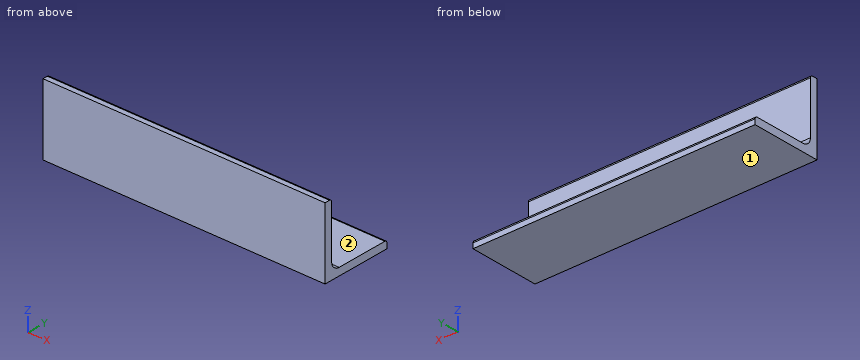
```python
from build123d import *

# Parameters (mm, degrees)
BASE_DEPTH = 300


with BuildPart() as part:
    # Sketch1 → Base (new body)
    with BuildSketch(Plane.YZ):
        with BuildLine():
            Line((0, 75), (0, 0))
            Line((0, 0), (75, 0))
            Line((75, 0), (75, 5.333333333))
            ThreePointArc((75, 5.333333333), (74.218951416, 7.218951416), (72.333333333, 8))
            Line((72.333333333, 8), (17, 8))
            ThreePointArc((17, 8), (10.636038969, 10.636038969), (8, 17))
            Line((8, 17), (8, 72.333333333))
            ThreePointArc((8, 72.333333333), (7.218951416, 74.218951416), (5.333333333, 75))
            Line((5.333333333, 75), (0, 75))
        make_face()
    extrude(amount=BASE_DEPTH)


solid = part.part
```
Geometry check sheet. Reference: the model listing, model coordinates, mm. Face numbers are marked on the shaded views. A direction names the side the tool comes from. Coordinates: 2 decimals unless noted, no trailing zeros. Loops run counter-clockwise (first coordinate to the right, second up) from the corner with the lowest first, then second, coordinate; pieces in that order, holes last. Notation, with made-up numbers: (61.25, 64.5) -> (87.25, 64.5) arc R16 cw to (87.25, 74.5) -> close; hole circle Ø9 at (48, -3). An arc over 180 degrees is marked (long way). Put each result on its own line as item: value.
1) Gauge pin test, flat ends, axial feed: pin 1 Ø5 at (x, z) = (50.5, 66.5) entering from +Y; pin 2 Ø12 at (y, z) = (14.5, 40) entering from +X. Record the tip position at first contact, or that the pin passes through.
Result set:
pin 1: stops at y = 8
pin 2: passes through
2) Cross-section at B-B on z = 63. Record the boundary of the cut face in (x, y), plus the area to 3 significant figures.
Result set:
outline: (0, 0) -> (300, 0) -> (300, 8) -> (0, 8) -> close
area: 2,400 mm^2
3) Tool access check on the marked faces 1 and 2. Record the directions out of +Z, -Z, +X, -X, +Y, -Y that give a thin tool (end or side, any length) a straight path to the whole face; none if there is none.
Result set:
face 1: -Z, +X, -X, +Y, -Y
face 2: +Z, +X, -X, +Y
4) Thickness scan on line 1 (Z direction, x = 95, y = 53.5); line 2 (Y direction, x = 210.5, z = 10.5). Record the ranges inside material, lowest first.
Result set:
line 1: z = 0 to 8
line 2: y = 0 to 10.78
5) Cross-section at A-A on x = 203.5. Record the boundary of the cut face in (y, z).
Result set:
outline: (0, 0) -> (75, 0) -> (75, 5.33) arc R2.67 ccw to (72.33, 8) -> (17, 8) arc R9 cw to (8, 17) -> (8, 72.33) arc R2.67 ccw to (5.33, 75) -> (0, 75) -> close
